Verification items for the finished model (mm, model axes). Face numbers are marked on the shaded views. A direction names the side the tool comes from. Coordinates: 2 decimals unless noted, no trailing zeros. Order: outer loops, then holes, each group sorted by start corner. A loop starts at its lowest first (then second) coordinate and runs counter-clockwise, first axis right, second up. Notation, with made-up numbers: M 51.25,22.5 L 80.25,22.5 A16 cw 80.25,46.5 Z; hole C 32,-30.75 d8. An arc over 180 degrees is marked long. Return JSON: item names as keys, results as strings. Group by question number.
1. Gauge pin test, flat ends, axial feed: pin 1 (3 mm diameter, centred on x = -13.5, z = 166, fed in from -Y); pin 2 (3 mm diameter, centred on x = 23.5, y = -18, fed in from +Z); pin 3 (2 mm diameter, centred on y = -22.5, z = 233, fed in from +X). Record the tip position at first contact, or that the pin passes through.
2. Section check D-D, the plane x = -34.5. Record the cut outline in (y, z), plus the area to 3 significant figures.
3. Set-up check for the marked faces 4, 5 and 6: record each of +Z, -Z, +X, -X, +Y, -Y from which the full face is reachable in a straight line by a thin tool's end or side.
4. Section check C-C, the plane z = 274. Record the cut outline in (x, y).
5. Section check A-A, the plane x = 0. Record the cut outline in (y, z).
6. Mould release check, pull along Z, two halves, no side actions. Record for the marked faces 1, 2 and 3: +Z half, -Z half, draft (parallel to the pull), parting line (faces both ways), or undercut.
7. Material ranges on line 1 along Y through (x, z) = (1.5, 105.5); line 2 along Z through (x, y) = (10, -30); line 3 along Z through (x, y) = (46, 6), recorded low to high.
```python
from build123d import *

# Parameters (mm, degrees)
SKETCH1_R           = 30
BOSS_EXTRUDE1_DEPTH = 28
SKETCH2_R           = 37.5
BOSS_EXTRUDE2_DEPTH = 53
SKETCH3_R           = 51.9465
BOSS_EXTRUDE3_DEPTH = 80
SKETCH4_R           = 37.5
BOSS_EXTRUDE4_DEPTH = 53
SKETCH5_R           = 30
BOSS_EXTRUDE5_DEPTH = 55
SKETCH6_R           = 24
BOSS_EXTRUDE6_DEPTH = 31


with BuildPart() as part:
    # Sketch1 → Boss-Extrude1 (new body)
    with BuildSketch(Plane.XY):
        Circle(SKETCH1_R)
    extrude(amount=BOSS_EXTRUDE1_DEPTH)

    # Sketch2 → Boss-Extrude2 (add)
    with BuildSketch(Plane.XY.offset(28)):
        Circle(SKETCH2_R)
    extrude(amount=BOSS_EXTRUDE2_DEPTH)

    # Sketch3 → Boss-Extrude3 (add)
    with BuildSketch(Plane.XY.offset(81)):
        Circle(SKETCH3_R)
    extrude(amount=BOSS_EXTRUDE3_DEPTH)

    # Sketch4 → Boss-Extrude4 (add)
    with BuildSketch(Plane.XY.offset(161)):
        Circle(SKETCH4_R)
    extrude(amount=BOSS_EXTRUDE4_DEPTH)

    # Sketch5 → Boss-Extrude5 (add)
    with BuildSketch(Plane.XY.offset(214)):
        Circle(SKETCH5_R)
    extrude(amount=BOSS_EXTRUDE5_DEPTH)

    # Sketch6 → Boss-Extrude6 (add)
    with BuildSketch(Plane.XY.offset(269)):
        Circle(SKETCH6_R)
    extrude(amount=BOSS_EXTRUDE6_DEPTH)


solid = part.part
```
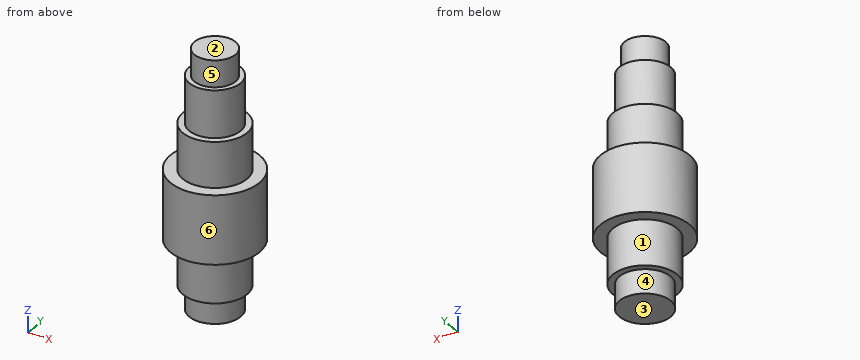
Answers follow:
{
 "1": {"pin 1": "y = -35.53", "pin 2": "z = 269", "pin 3": "x = 20.92"},
 "2": {"outline": "M -38.84,81 L -14.7,81 L -14.7,28 L 14.7,28 L 14.7,81 L 38.84,81 L 38.84,161 L 14.7,161 L 14.7,214 L -14.7,214 L -14.7,161 L -38.84,161 Z", "area": "9,330 mm^2"},
 "3": {"face 4": "-Z", "face 5": "+Z", "face 6": "+Z, -Z"},
 "4": {"outline": "C 0,0 d48"},
 "5": {"outline": "M -51.95,81 L -37.5,81 L -37.5,28 L -30,28 L -30,0 L 30,0 L 30,28 L 37.5,28 L 37.5,81 L 51.95,81 L 51.95,161 L 37.5,161 L 37.5,214 L 30,214 L 30,269 L 24,269 L 24,300 L -24,300 L -24,269 L -30,269 L -30,214 L -37.5,214 L -37.5,161 L -51.95,161 Z"},
 "6": {"face 1": "draft", "face 2": "+Z half", "face 3": "-Z half"},
 "7": {"line 1": "-51.92 to 51.92", "line 2": "28 to 214", "line 3": "81 to 161"}
}
